The listing builds one solid part. Answer for the finished solid, in the listing's coordinates (mm). A direction names the side the tool comes from. Round coordinates to 2 decimals unless told otherwise and drop trailing zeros. Write each loop counter-clockwise with the first axis right and the second up, starting at its lowest first coordinate (ties: lowest second). Pieces come first, ordered by that corner, then holes. Notation, with made-up numbers: (-15.75, 63) - (16.25, 63) arc R23 cw to (16.25, 90) - close; hole circle Ø7 at (75.5, -14). An arc over 180 degrees is marked (long way). Use a Markdown table: item, result. Add a question column.
1) A cutting plane is placed at A-A (y = -1). Give the vertices of the cut face in (x, z).
2) A cutting plane is placed at C-C (x = 2.15). Give the vertices of the cut face in (y, z), then the cut area to 3 significant figures.
3) A cutting plane is placed at B-B (z = -1.25). Give the vertices of the cut face in (x, y), then the cut area to 4 significant figures.
4) Determine the mould class of faces 3 (the flat face through (1, 1, 12.5)), 4 (the flat face through (0, 15, 0)), 5 (the flat face through (1, 0, -9.6)), 6 (the flat face through (1, 29.25, 0)) for opening direction Z: +Z half, -Z half, draft (parallel to the pull), parting line (faces both ways), or undercut.
5) This flat-tipped pin is pushed along its axis until it touches: P1, Ø1, axis at x = 0.5, y = 22, coming from the +Z side. Where does it stop, or does it pass through?
6) A cutting plane is placed at D-D (z = -7.5). Give the vertices of the cut face in (x, y), then the cut area to 3 significant figures.
7) Find the intervals of material crossed by probe 1 along Z at (x, y) = (0.85, -1); probe 2 along Y at (x, z) = (0.15, -0.5); probe 3 along Z at (x, y) = (2.55, 33.5), in increasing order. Write a range as from..to.
8) A tool of negligible diameter and unlimited length cuts with its end or side. For faces 1 (the flat face through (3, 15, 0)), 2 (the cylindrical face through (1.48, 31.55, 4.75)), from which of +Z, -Z, +X, -X, +Y, -Y can it reach the whole face along a straight path? Write none if from no direction.
```python
from build123d import *

# Parameters (mm, degrees)
EXTRUDE_1_DEPTH             = 3
EXTRUDE_2_DEPTH             = 3
FILLET_1_R                  = 2
CUT_EXTRUDE_1_DEPTH         = 3
FILLET_2_R                  = 2
HOLE_WIZARD_4_3_4_3_1_D     = 4.3
HOLE_WIZARD_4_3_4_3_1_DEPTH = 10.1
HOLE_WIZARD_4_3_4_3_1_TIP   = 1.291850331
SKETCH_7_W                  = 24.449376322
SKETCH_7_H                  = 27.885292322
CUT_EXTRUDE_2_DEPTH         = 10
CUT_EXTRUDE_3_DEPTH         = 10
FILLET_3_R                  = 5


with BuildPart() as part:
    # 草图1 → 凸台-拉伸1 (new body)
    with BuildSketch(Plane(origin=(0, 0, 0), x_dir=(0, 0, -1), z_dir=(1, 0, 0))):
        Polygon((-12.5, 6), (-6, 6), (-6, 61), (6, 61), (6, 6), (12.5, 6), (12.5, -6), (-12.5, -6), align=None)
    extrude(amount=EXTRUDE_1_DEPTH)

    # 草图2 → 凸台-拉伸2 (add)
    with BuildSketch(Plane.ZY):
        Polygon((-6, 61), (-12.5, 6), (12.5, 6), (6, 61), align=None)
    extrude(amount=-EXTRUDE_2_DEPTH)

    # 圆角1
    fillet_1_edges = [part.edges().sort_by_distance(p)[0] for p in [
        (1.5, 61, 6),
        (1.5, 61, -6),
    ]]
    fillet(fillet_1_edges, radius=FILLET_1_R)

    # 草图3 → 切除-拉伸1 (cut)
    with BuildSketch(Plane.ZY):
        with BuildLine():
            Line((-5.4, 2), (-5.4, -2))
            ThreePointArc((-5.4, -2), (-7.5, -4.1), (-9.6, -2))
            Line((-9.6, -2), (-9.6, 2))
            ThreePointArc((-9.6, 2), (-7.5, 4.1), (-5.4, 2))
        make_face()
        with BuildLine():
            Line((5.4, 2), (5.4, -2))
            ThreePointArc((5.4, -2), (7.5, -4.1), (9.6, -2))
            Line((9.6, -2), (9.6, 2))
            ThreePointArc((9.6, 2), (7.5, 4.1), (5.4, 2))
        make_face()
    extrude(amount=-CUT_EXTRUDE_1_DEPTH, mode=Mode.SUBTRACT)

    # 圆角2
    fillet_2_edges = [part.edges().sort_by_distance(p)[0] for p in [
        (1.5, -6, -12.5),
        (1.5, -6, 12.5),
    ]]
    fillet(fillet_2_edges, radius=FILLET_2_R)

    # Ø4.3 (4.3) 直径孔1
    with Locations(Plane.ZY):
        with Locations((0, 56), (0, 41)):
            Hole(HOLE_WIZARD_4_3_4_3_1_D / 2, depth=HOLE_WIZARD_4_3_4_3_1_DEPTH)
            with Locations((0, 0, -(HOLE_WIZARD_4_3_4_3_1_DEPTH + HOLE_WIZARD_4_3_4_3_1_TIP / 2))):  # 118° drill point
                Cone(0, HOLE_WIZARD_4_3_4_3_1_D / 2, HOLE_WIZARD_4_3_4_3_1_TIP, mode=Mode.SUBTRACT)

    # 草图7 → 切除-拉伸2 (cut)
    with BuildSketch(Plane(origin=(3, 0, 0), x_dir=(0, 0, -1), z_dir=(1, 0, 0))):
        with Locations((-1.251346032, 49.942646161)):
            Rectangle(SKETCH_7_W, SKETCH_7_H)
    extrude(amount=-CUT_EXTRUDE_2_DEPTH, mode=Mode.SUBTRACT)

    # 草图8 → 切除-拉伸3 (cut)
    with BuildSketch(Plane.ZY):
        with BuildLine():
            Line((-2.5, 33.75), (2.5, 33.75))
            ThreePointArc((2.5, 33.75), (4.75, 31.5), (2.5, 29.25))
            Line((2.5, 29.25), (-2.5, 29.25))
            ThreePointArc((-2.5, 29.25), (-4.75, 31.5), (-2.5, 33.75))
        make_face()
    extrude(amount=-CUT_EXTRUDE_3_DEPTH, mode=Mode.SUBTRACT)

    # 圆角3
    fillet_3_edges = [part.edges().sort_by_distance(p)[0] for p in [
        (1.5, 36, 8.954545455),
        (1.5, 36, -8.954545455),
    ]]
    fillet(fillet_3_edges, radius=FILLET_3_R)


solid = part.part
```
Entries:
| question | item | result |
|---|---|---|
| 1 | outline | (0, -12.5) - (3, -12.5) - (3, -9.6) - (0, -9.6) - close; (0, -5.4) - (3, -5.4) - (3, 5.4) - (0, 5.4) - close; (0, 9.6) - (3, 9.6) - (3, 12.5) - (0, 12.5) - close |
| 2 | outline | (-6, -10.5) arc R2 ccw to (-4, -12.5) - (6, -12.5) - (31.59, -9.48) arc R5 ccw to (36, -4.51) - (36, 4.51) arc R5 ccw to (31.59, 9.48) - (6, 12.5) - (-4, 12.5) arc R2 ccw to (-6, 10.5) - close; hole (-2, -9.6) - (2, -9.6) arc R2.1 ccw to (2, -5.4) - (-2, -5.4) arc R2.1 ccw to start; hole (-2, 5.4) - (2, 5.4) arc R2.1 ccw to (2, 9.6) - (-2, 9.6) arc R2.1 ccw to start; hole (29.25, -2.5) arc R2.25 ccw to (33.75, -2.5) - (33.75, 2.5) arc R2.25 ccw to (29.25, 2.5) - close |
| 2 | area | 834 mm² |
| 3 | outline | (0, -6) - (3, -6) - (3, 29.25) - (0, 29.25) - close; (0, 33.75) - (3, 33.75) - (3, 36) - (0, 36) - close |
| 3 | area | 112.5 mm² |
| 4 | face 3 | +Z half |
| 4 | face 4 | draft |
| 4 | face 5 | undercut |
| 4 | face 6 | undercut |
| 5 | P1 | stops at z = 10.67 |
| 6 | outline | (0, -6) - (3, -6) - (3, -4.1) - (0, -4.1) - close; (0, 4.1) - (3, 4.1) - (3, 35.01) - (0, 35.01) - close |
| 6 | area | 98.4 mm² |
| 7 | probe 1 | z = -12.5..-9.6, -5.4..5.4, 9.6..12.5 |
| 7 | probe 2 | y = -6..29.25, 33.75..36 |
| 7 | probe 3 | z = -8.84..-3.53, 3.53..8.84 |
| 8 | face 1 | +Z, -Z, +X, +Y, -Y |
| 8 | face 2 | +X, -X |
